Can you work these out from the drawing? Everything is in mm from the part's minimum corner. A direction names the side the tool comes from. Round coordinates to 2 decimals unless told otherwise and drop trailing zeros. Loops run counter-clockwise (first coordinate to the right, second up) from the corner with the lowest first, then second, coordinate; pieces in that order, holes last. Notation, with made-up numbers: M 49.25,10.25 L 85.25,10.25 A8 cw 85.25,18.25 Z; hole C 45.5,-27 d10. An arc over 180 degrees is marked long. Use a Markdown table: item, result.
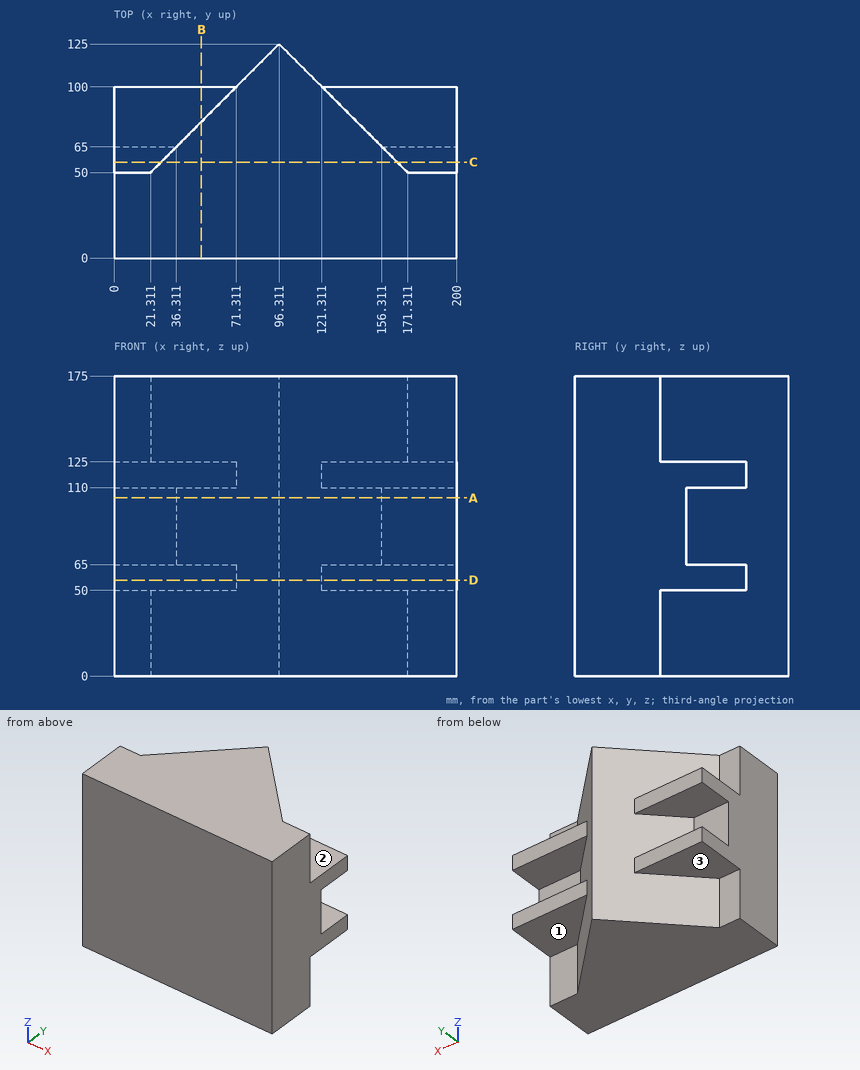
1. Imagine slicing it at A-A, the plane z = 104. Write out the boundary of the cut face in (x, y), then the cut area to 3 significant figures.
Answer sheet:
| item | result |
|---|---|
| outline | M 0,0 L 200,0 L 200,65 L 156.31,65 L 96.31,125 L 36.31,65 L 0,65 Z |
| area | 16,600 mm2 |
2. For pin 1 Ø10.5 at (x, y) = (155.5, 85.5) entering from +Z; pin 2 Ø10.5 at (x, y) = (159.5, 79) entering from -Z; pin 3 Ø12 at (x, z) = (51, 59.5) entering from +Y, each with a flat end and sliding along its axis, tell me the tip position at first contact or that it passes through.
Answer sheet:
| item | result |
|---|---|
| pin 1 | z = 125 |
| pin 2 | z = 50 |
| pin 3 | y = 100 |
3. Imagine slicing it at D-D, the plane z = 56. Write out the boundary of the cut face in (x, y), then the cut area to 3 significant figures.
Answer sheet:
| item | result |
|---|---|
| outline | M 0,0 L 200,0 L 200,100 L 121.31,100 L 96.31,125 L 71.31,100 L 0,100 Z |
| area | 20,600 mm2 |
4. Imagine slicing it at C-C, the plane y = 56. Write out the boundary of the cut face in (x, z), then the cut area to 3 significant figures.
Answer sheet:
| item | result |
|---|---|
| outline | M 0,50 L 27.31,50 L 27.31,0 L 165.31,0 L 165.31,50 L 200,50 L 200,125 L 165.31,125 L 165.31,175 L 27.31,175 L 27.31,125 L 0,125 Z |
| area | 28,800 mm2 |
5. I need wall thicknesses on probe 1 along Z at (x, y) = (164.5, 89.5); probe 2 along Y at (x, z) = (11.5, 24.5); probe 3 along X at (y, z) = (85.5, 20.5). Which ranges of each line are inside material? Lowest first, please. Write a range as from..to.
Answer sheet:
| item | result |
|---|---|
| probe 1 | 50..65, 110..125 |
| probe 2 | 0..50 |
| probe 3 | 56.81..135.81 |
6. Which directions (+Z, -Z, +X, -X, +Y, -Y) give clear straight access to the entire face, cutting with the end or side of a thin tool? Please do the marked faces 1, 2 and 3.
Answer sheet:
| item | result |
|---|---|
| face 1 | -Z, +X, +Y |
| face 2 | +Z, +X, +Y |
| face 3 | -Z, -X, +Y |
7. Imagine slicing it at B-B, the plane x = 51. Write out the boundary of the cut face in (y, z).
Answer sheet:
| item | result |
|---|---|
| outline | M 0,0 L 79.69,0 L 79.69,50 L 100,50 L 100,65 L 79.69,65 L 79.69,110 L 100,110 L 100,125 L 79.69,125 L 79.69,175 L 0,175 Z |
